Could you check a few things on this model? Use its own coordinates, in mm. Give positions to 0.01 mm unless a question says otherwise; leave off trailing zeros. Loops run counter-clockwise (first coordinate to the right, second up) from the corner with the lowest first, then second, coordinate; pieces in that order, holes last. Notation, with made-up numbers: (-20.5, 71) -> (35.5, 71) arc R21 cw to (35.5, 82) -> close; hole circle Ø8 at (26.25, 37.5). An arc over 180 degrees is marked (long way). Write each question's results on one line, items separated by ' | '. Start each with the question number.
Q1. If we section it at A-A, the plane x = 84: List the corners of the cut face in (y, z) for me.
Q2. We'd pull the mould along X, two halves only. Please class faces 1 (the face through (89, 1, -50)), 2 (the face through (143.65, 0.51, -0.86)), 3 (the face through (84.481, 0.493, -109.474)): released by +X, released by -X, zero draft, split by the parting line, or undercut.
Q3. If we section it at D-D, the plane x = 54.55: List the corners of the cut face in (y, z) for me, plus the area to 3 significant figures.
Q4. If I drill on line 1 along X through (y, z) = (0.7, -6); line 2 along X through (y, z) = (0.8, -111); line 3 along Z through (x, y) = (74, 0.7), over which ranges is the centre line in solid material (lowest first)?
Q5. If we section it at B-B, the plane z = -111: List the corners of the cut face in (x, y) for me, plus the area to 4 significant figures.
Q6. Will these pins go through, and if not, where does the flat tip stop? P1, Ø3, axis at x = 84, z = -111, coming from the -Y side; P2, Ø4, axis at x = 95.5, z = -82, coming from the -Y side.
Q7. If we section it at C-C, the plane y = 0.65: List the corners of the cut face in (x, z) for me.
from build123d import *

# Parameters (mm, degrees)
SKETCH_1_R      = 1.6
EXTRUDE_1_DEPTH = 1
FILLET_1_R      = 3


with BuildPart() as part:
    # 草图1 → 凸台-拉伸1 (new body)
    with BuildSketch(Plane(origin=(0, 0, 0), x_dir=(1, 0, 0), z_dir=(0, 1, 0))):
        Polygon((0, 0), (0, 72), (69, 78.5), (69, 127), (144.55, 127), (144.55, 0), align=None)
        with Locations(Location((74, 111, 0), (0, 0, 270))):
            Circle(SKETCH_1_R, mode=Mode.SUBTRACT)
        with Locations(Location((84, 111, 0), (0, 0, 270))):
            Circle(SKETCH_1_R, mode=Mode.SUBTRACT)
        with Locations(Location((34.55, 6, 0), (0, 0, 270))):
            Circle(SKETCH_1_R, mode=Mode.SUBTRACT)
        with Locations(Location((54.55, 6, 0), (0, 0, 270))):
            Circle(SKETCH_1_R, mode=Mode.SUBTRACT)
    extrude(amount=EXTRUDE_1_DEPTH)

    # 圆角1
    fillet_1_edges = [part.edges().sort_by_distance(p)[0] for p in [
        (0, 0.5, 0),
        (0, 0.5, -72),
        (69, 0.5, -78.5),
        (69, 0.5, -127),
        (144.55, 0.5, -127),
        (144.55, 0.5, 0),
    ]]
    fillet(fillet_1_edges, radius=FILLET_1_R)


solid = part.part
Final values:
1) outline: (0, -127) -> (1, -127) -> (1, -112.6) -> (0, -112.6) -> close; (0, -109.4) -> (1, -109.4) -> (1, 0) -> (0, 0) -> close
2) face 1: zero draft | face 2: released by +X | face 3: undercut
3) outline: (0, -77.14) -> (1, -77.14) -> (1, -7.6) -> (0, -7.6) -> close; (0, -4.4) -> (1, -4.4) -> (1, 0) -> (0, 0) -> close | area: 73.9 mm²
4) line 1: x = 0 to 32.95, 36.15 to 52.95, 56.15 to 144.55 | line 2: x = 69 to 72.4, 75.6 to 82.4, 85.6 to 144.55 | line 3: z = -127 to -112.6, -109.4 to 0
5) outline: (69, 0) -> (72.4, 0) -> (72.4, 1) -> (69, 1) -> close; (75.6, 0) -> (82.4, 0) -> (82.4, 1) -> (75.6, 1) -> close; (85.6, 0) -> (144.55, 0) -> (144.55, 1) -> (85.6, 1) -> close | area: 69.15 mm²
6) P1: passes through | P2: stops at y = 0
7) outline: (0, -69.27) arc R3 ccw to (2.72, -72.26) -> (66.28, -78.24) arc R3 cw to (69, -81.23) -> (69, -124) arc R3 ccw to (72, -127) -> (141.55, -127) arc R3 ccw to (144.55, -124) -> (144.55, -3) arc R3 ccw to (141.55, 0) -> (3, 0) arc R3 ccw to (0, -3) -> close; hole circle Ø3.2 at (34.55, -6); hole circle Ø3.2 at (54.55, -6); hole circle Ø3.2 at (74, -111); hole circle Ø3.2 at (84, -111)
